Could you check a few things on this model? Use its own coordinates, in mm. Coordinates: 2 decimals unless noted, no trailing zeros. Loops run counter-clockwise (first coordinate to the right, second up) from the corner with the lowest first, then second, coordinate; pieces in that order, holes last. Notation, with made-up numbers: (56.25, -21) - (77.25, -21) arc R16 cw to (77.25, -1) - close; hole circle Ø3 at (-8, 61). An arc over 180 degrees is marked (long way). One line per item, written item: value. Start each with the question number.
(1) If we section it at B-B on z = 240: Write out the boundary of the cut face in (x, y), then the cut area to 3 significant figures.
(2) If I drill on line 1 along Z through (x, y) = (0, 3.5); line 2 along Z through (x, y) = (0, 2); line 3 along Z through (x, y) = (-1.75, -3), over which ranges is the centre line in solid material (lowest first)? Write a range as from..to.
(3) I'm going to push flat-ended pins straight in: P1, Ø1, axis at x = 0, z = 283, coming from the +Y side; P2, Ø5, axis at x = -5.5, z = 291.5, coming from the +Y side; P3, Ø3, axis at x = 2, z = 316, coming from the -Y side. Where does each tip first touch, or does it pass through?
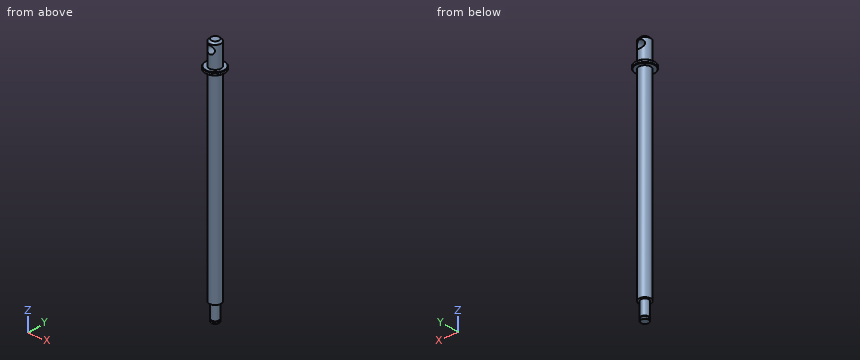
```python
from build123d import *

# Parameters (mm, degrees)
SKETCH4_R          = 4
CUT_EXTRUDE2_DEPTH = 25
CHAMFER2_SIZE      = 2
CHAMFER3_SIZE      = 0.2
SKETCH5_R          = 10
BOSS_EXTRU_1_DEPTH = 3
CHAMFER4_SIZE      = 0.5


with BuildPart() as part:
    # Sketch1 → Revolve1 (revolve)
    with BuildSketch(Plane(origin=(0, 0, 0), x_dir=(1, 0, 0), z_dir=(0, 1, 0)), mode=Mode.PRIVATE) as revolve1_sk:
        Polygon((4.142447891, -208.268648203), (3.342447891, -208.268648203), (3.342447891, -209.168648203), (4.142447891, -209.168648203), (4.142447891, -224.268648203), (6.142447891, -224.268648203), (6.142447891, -456.268648203), (0.142447891, -456.268648203), (0.142447891, -206.268648203), (4.142447891, -206.268648203), align=None)
    revolve(revolve1_sk.sketch.rotate(Axis((0.142447891, 0, 206.268648203), (0, 0, 1)), 180), axis=Axis((0.142447891, 0, 206.268648203), (0, 0, 1)))

    # Sketch4 → Cut-Extrude2 (cut, symmetric)
    with BuildSketch(Plane(origin=(0, 0, 0), x_dir=(1, 0, 0), z_dir=(0, 1, 0))):
        with Locations(Location((0, -448.894244445, 0), (0, 0, 270))):
            Circle(SKETCH4_R)
    extrude(amount=CUT_EXTRUDE2_DEPTH, both=True, mode=Mode.SUBTRACT)

    # Chamfer2
    chamfer2_edges = [part.edges().sort_by_distance(p)[0] for p in [
        (6.142447891, 0, 456.268648203),
    ]]
    chamfer(chamfer2_edges, length=CHAMFER2_SIZE)

    # Chamfer3
    chamfer3_edges = [part.edges().sort_by_distance(p)[0] for p in [
        (4.142447891, 0, 206.268648203),
    ]]
    chamfer(chamfer3_edges, length=CHAMFER3_SIZE)

    # Sketch5 → Boss.-Extru.1 (add)
    with BuildSketch(Plane.XY.offset(429.268648203)):
        Circle(SKETCH5_R)
    extrude(amount=BOSS_EXTRU_1_DEPTH)

    # Chamfer4
    chamfer4_edges = [part.edges().sort_by_distance(p)[0] for p in [
        (-10, 0, 429.268648203),
        (-10, 0, 432.268648203),
    ]]
    chamfer(chamfer4_edges, length=CHAMFER4_SIZE)


solid = part.part
```
Values:
1. outline: circle Ø12 at (0.14, 0)
1. area: 113 mm2
2. line 1: z = 206.27..208.27, 209.17..444.89, 452.89..456.27
2. line 2: z = 206.27..444.89, 452.89..456.27
2. line 3: z = 206.27..208.27, 209.17..445.3, 452.49..456.27
3. P1: stops at y = 6
3. P2: stops at y = 5.11
3. P3: stops at y = -5.99
